Geometry: see drawing. Coordinates: mm, zero at the bounding-box minimum. A direction names the side the tool comes from. Coordinates: 2 decimals unless noted, no trailing zeros. Loops run counter-clockwise (first coordinate to the right, second up) from the corner with the lowest first, then second, coordinate; pieces in that order, holes last. Notation, with made-up numbers: (57, 43.25) - (107, 43.25) arc R30 ccw to (107, 69.25) - close; hole circle Ø9 at (74.25, 16). An arc over 180 degrees is marked (long way). Write item = value, one per line. Start each with the question number.
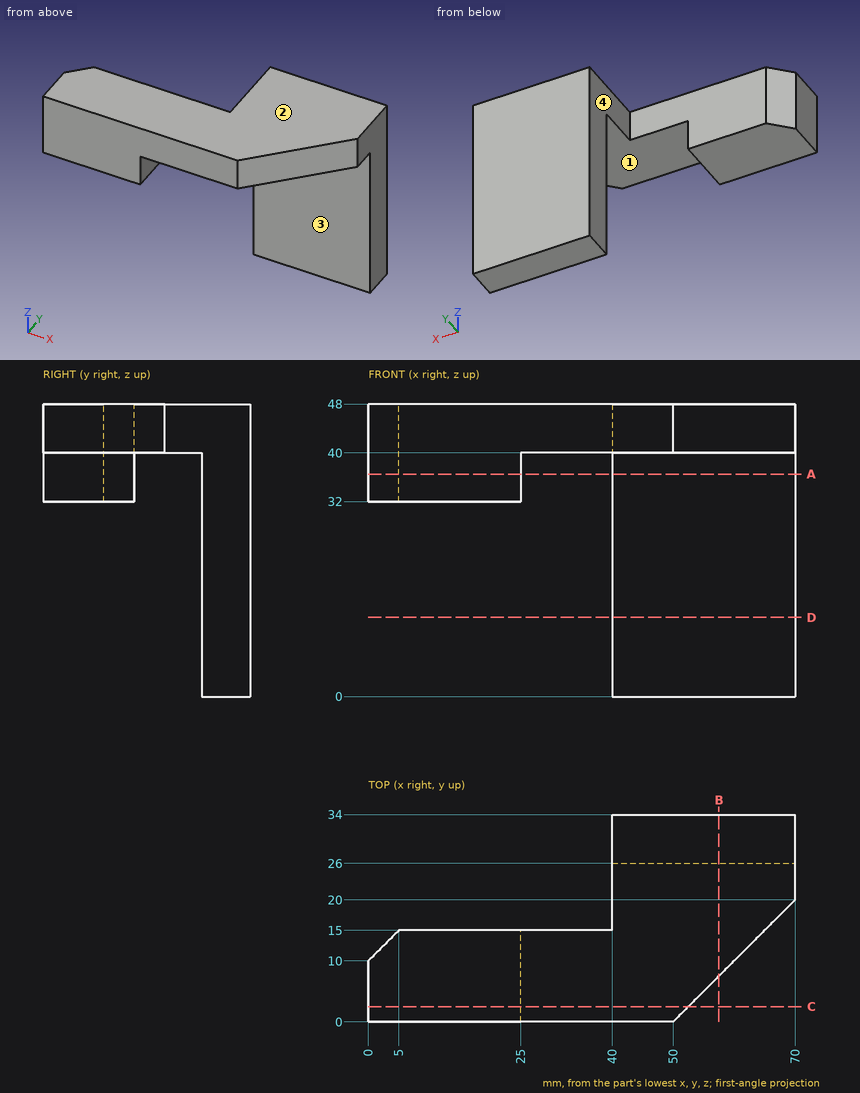
Item 1: Cut plane B-B (x = 57.5). Return the cut outline in (y, z), then the cut area to 3 significant figures.
Item 2: Cut plane C-C (y = 2.5). Return the cut outline in (x, z).
Item 3: Material intervals for L1, parallel to Z at x = 13.5, y = 9.5; L2, parallel to Z at x = 67.5, y = 19; L3, parallel to X at y = 32.5, z = 28, sorted ascending. Write a range as [from, to].
Item 4: Cut plane D-D (z = 13). Return the cut outline in (x, y).
Item 5: Cut plane A-A (z = 36.5). Return the cut outline in (x, y).
Item 6: First-contact query: pin 1 (7.5 mm diameter, centred on x = 17.5, y = 8, fed in from -Z); pin 2 (13 mm diameter, centred on x = 53.5, y = 17.5, fed in from -Z); pin 3 (13 mm diameter, centred on x = 18, z = 42, fed in from +Y). Flat tips, straight axial feed; report the tip coordinate or a pass-through.
Item 7: Reachability of the marked faces 1, 2, 3 and 4 from +Z, -Z, +X, -X, +Y, -Y: full face, straight path, thin tool, end or side. Return the list, or none.
Responses:
q1.outline = (7.5, 40) - (26, 40) - (26, 0) - (34, 0) - (34, 48) - (7.5, 48) - close
q1.area = 532 mm2
q2.outline = (0, 32) - (25, 32) - (25, 40) - (52.5, 40) - (52.5, 48) - (0, 48) - close
q3.L1 = [32, 48]
q3.L2 = [40, 48]
q3.L3 = [40, 70]
q4.outline = (40, 26) - (70, 26) - (70, 34) - (40, 34) - close
q5.outline = (0, 0) - (25, 0) - (25, 15) - (5, 15) - (0, 10) - close; (40, 26) - (70, 26) - (70, 34) - (40, 34) - close
q6.pin_1 = 32
q6.pin_2 = 40
q6.pin_3 = 15
q7.face_1 = -Z, +X, -Y
q7.face_2 = +Z, +X, -X, +Y, -Y
q7.face_3 = -Z, +X, -X, -Y
q7.face_4 = +Z, -Z, -X, +Y
